Geometry: final body of the model. Coordinates: model frame, mm. Face numbers are marked on the shaded views. A direction names the side the tool comes from. Give positions to 0.01 mm unless a question says otherwise; leave off trailing zeros. Order: outer loops, then holes, each group sorted by start corner. A loop starts at its lowest first (then second) coordinate and runs counter-clockwise, first axis right, second up. Notation, with made-up numbers: (-27.5, 19) -> (-18.5, 19) arc R14 ccw to (-18.5, 30) -> close; hole circle Ø7 at (-39.75, 7.5). An arc over 180 degrees is marked (long way). Answer in a Markdown table with one row per item. Add a question column.
Q1. Cut plane A-A on z = 10. Return the cut outline in (x, y), and give its area (3 significant figures).
Q2. Cut plane D-D on z = 1. Return the cut outline in (x, y), and give its area (3 significant figures).
Q3. Cut plane C-C on y = 0. Return the cut outline in (x, z), and give its area (3 significant figures).
Q4. Cut plane B-B on z = -1.5. Return the cut outline in (x, y), and give its area (3 significant figures).
Q5. Contact query for flat-ended pins moving along their axis: P1, Ø1.5, axis at x = -1.5, y = -15, coming from the +Z side; P2, Ø4.5, axis at x = 0.5, y = 6, coming from the -Z side; P3, Ø2.5, axis at y = -36.5, z = -5.5, coming from the +X side. Output: stop coordinate, or through.
Q6. Set-up query: the marked faces 1, 2, 3, 4 and 5. Return all of +Z, -Z, +X, -X, +Y, -Y with unobstructed straight access to the full face (end or side cutting, diameter ignored); none if empty.
Q7. Pull-direction query (X, two-part tool) for the marked faces 6, 7, 8 and 9; classes: +X half, -X half, draft (parallel to the pull), parting line (faces both ways), or undercut.
Q8. Line query: line 1 along Y through (x, z) = (0, 5); line 2 along Y through (x, z) = (0, 1.5); line 3 along Z through (x, y) = (1.75, 3). Output: solid intervals per line, ascending. Write a range as from..to.
from build123d import *

# Parameters (mm, degrees)
EXTRUDE_1_DEPTH      = 8
EXTRUDE_1_DEPTH_BACK = 8
SKETCH_2_W           = 16
SKETCH_2_H           = 10
CUT_EXTRUDE_1_DEPTH  = 2.5
SKETCH_3_W           = 5
SKETCH_3_H           = 5.75
SKETCH_4_R           = 11.5
CUT_EXTRUDE_2_DEPTH  = 5
SKETCH_6_R           = 7
SKETCH_6_R_2         = 6.5
CUT_EXTRUDE_3_DEPTH  = 7
CUT_EXTRUDE_4_DEPTH  = 3.5


with BuildPart() as part:
    # 草图1 → 凸台-拉伸1 (new, two sides: drawn at the far end of the back side and taken through both)
    with BuildSketch(Plane(origin=(0, 0, 0), x_dir=(0, 0, -1), z_dir=(1, 0, 0)).offset(-EXTRUDE_1_DEPTH_BACK)):
        Polygon((-11.5, 9), (-11.5, -7.7), (-8.5, -42), (2.5, -42), (2.5, 9), align=None)
    extrude(amount=EXTRUDE_1_DEPTH + EXTRUDE_1_DEPTH_BACK)

    # 草图2 → 切除-拉伸1 (cut)
    with BuildSketch(Plane.XY):
        Rectangle(SKETCH_2_W, SKETCH_2_H)
    extrude(amount=-CUT_EXTRUDE_1_DEPTH, mode=Mode.SUBTRACT)

    # 草图3 → 旋转1 (revolve)
    with BuildSketch(Plane(origin=(0, 0, 0), x_dir=(0, 0, -1), z_dir=(1, 0, 0)), mode=Mode.PRIVATE) as revolve_1_sk:
        with Locations((5, -32.125)):
            Rectangle(SKETCH_3_W, SKETCH_3_H)
    revolve(revolve_1_sk.sketch.rotate(Axis((0, -35, -7.5), (0, 0, 1)), 270), axis=Axis((0, -35, -7.5), (0, 0, 1)))

    # 草图4 → 切除-拉伸2 (cut)
    with BuildSketch(Plane(origin=(0, 0, -7.5), x_dir=(-1, 0, 0), z_dir=(0, 0, -1))):
        with Locations((0, -35)):
            Circle(SKETCH_4_R)
        Polygon((0, -40.75), (4.979646072, -37.875), (4.979646072, -32.125), (0, -29.25), (-4.979646072, -32.125), (-4.979646072, -37.875), align=None, mode=Mode.SUBTRACT)
    extrude(amount=-CUT_EXTRUDE_2_DEPTH, mode=Mode.SUBTRACT)

    # 草图5 → 切除-旋转1 (revolve, cut)
    with BuildSketch(Plane(origin=(0, 0, 0), x_dir=(0, 0, -1), z_dir=(1, 0, 0)), mode=Mode.PRIVATE) as cut_revolve_1_sk:
        Polygon((-9.112244898, -35), (-9.374635569, -32), (-8.785774052, -32.5415), (6.9585, -32.5415), (7.5, -32), (7.5, -35), align=None)
    revolve(cut_revolve_1_sk.sketch.rotate(Axis((0, -35, -7.5), (0, 0, 1)), 270), axis=Axis((0, -35, -7.5), (0, 0, 1)), mode=Mode.SUBTRACT)

    # 草图6 → 切除-拉伸3 (cut)
    with BuildSketch(Plane.XY.offset(11.5)):
        Circle(SKETCH_6_R)
        Circle(SKETCH_6_R_2, mode=Mode.SUBTRACT)
    extrude(amount=-CUT_EXTRUDE_3_DEPTH, mode=Mode.SUBTRACT)

    # 草图7 → 切除-拉伸4 (cut)
    with BuildSketch(Plane.XY.offset(11.5)):
        Polygon((-3, 1.732050808), (-3, -1.732050808), (0, -3.464101615), (3, -1.732050808), (3, 1.732050808), (0, 3.464101615), align=None)
    extrude(amount=-CUT_EXTRUDE_4_DEPTH, mode=Mode.SUBTRACT)


solid = part.part
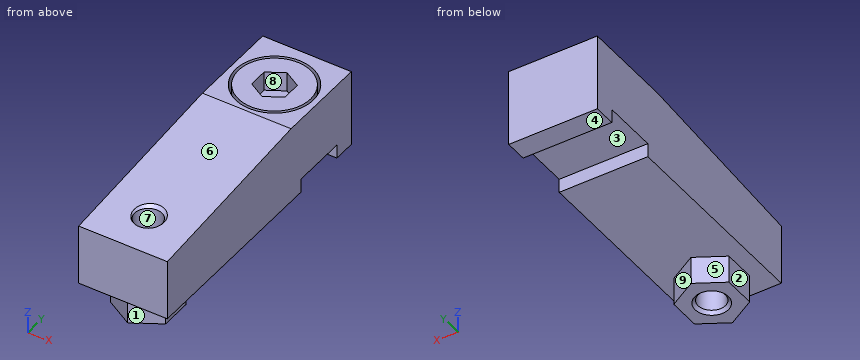
Completed:
| question | item | result |
|---|---|---|
| 1 | outline | (-8, -24.85) -> (8, -24.85) -> (8, 9) -> (-8, 9) -> close; circle Ø13 at (0, 0); hole circle Ø14 at (0, 0); hole (-3, -1.73) -> (0, -3.46) -> (3, -1.73) -> (3, 1.73) -> (0, 3.46) -> (-3, 1.73) -> close |
| 1 | area | 489 mm² |
| 2 | outline | (-8, -42) -> (8, -42) -> (8, 9) -> (-8, 9) -> close; hole circle Ø4.92 at (0, -35) |
| 2 | area | 797 mm² |
| 3 | outline | (-8, 0) -> (8, 0) -> (8, 11.5) -> (7, 11.5) -> (7, 4.5) -> (6.5, 4.5) -> (6.5, 11.5) -> (3, 11.5) -> (3, 8) -> (-3, 8) -> (-3, 11.5) -> (-6.5, 11.5) -> (-6.5, 4.5) -> (-7, 4.5) -> (-7, 11.5) -> (-8, 11.5) -> close |
| 3 | area | 156 mm² |
| 4 | outline | (-8, -42) -> (8, -42) -> (8, -5) -> (-8, -5) -> close; (-8, 5) -> (8, 5) -> (8, 9) -> (-8, 9) -> close; hole circle Ø4.92 at (0, -35) |
| 4 | area | 637 mm² |
| 5 | P1 | stops at z = 10.93 |
| 5 | P2 | stops at z = -2.5 |
| 5 | P3 | stops at x = 4.98 |
| 6 | face 1 | -Z, +X, -Y |
| 6 | face 2 | -Z, -X, +Y, -Y |
| 6 | face 3 | -Z, +X, -X |
| 6 | face 4 | -Z, +X, -X, +Y |
| 6 | face 5 | -Z, -X, +Y |
| 7 | face 6 | draft |
| 7 | face 7 | undercut |
| 7 | face 8 | undercut |
| 7 | face 9 | +X half |
| 8 | line 1 | y = -42..-37.46, -32.54..-7, -6.5..6.5, 7..9 |
| 8 | line 2 | y = -42..-37.46, -32.54..9 |
| 8 | line 3 | z = 0..11.5 |
